from build123d import *

# Parameters (mm, degrees)
EXTRUDE_1_DEPTH      = 0.5
EXTRUDE_1_DEPTH_BACK = 0.5
SKETCH_1_R           = 0.6


with BuildPart() as part:
    # 草图1 → 凸台-拉伸1 (new, two sides: drawn at the far end of the back side and taken through both)
    with BuildSketch(Plane(origin=(0, 0, 0), x_dir=(0, 0, -1), z_dir=(1, 0, 0)).offset(-EXTRUDE_1_DEPTH_BACK)):
        with BuildLine():
            Line((-1.575903864, -5.685642181), (-0.792131706, -4.328108982))
            ThreePointArc((-0.792131706, -4.328108982), (-1.835210176, -2.355544978), (-3.685531471, -3.602674702))
            ThreePointArc((-3.685531471, -3.602674702), (0, 4.4), (3.685531471, -3.602674702))
            ThreePointArc((3.685531471, -3.602674702), (1.835210176, -2.355544978), (0.792131706, -4.328108982))
            Line((0.792131706, -4.328108982), (1.575903864, -5.685642181))
            ThreePointArc((1.575903864, -5.685642181), (0, 5.9), (-1.575903864, -5.685642181))
        make_face()
        with Locations((2.2, -3.810511777)):
            Circle(SKETCH_1_R, mode=Mode.SUBTRACT)
        with Locations((-2.2, -3.810511777)):
            Circle(SKETCH_1_R, mode=Mode.SUBTRACT)
    extrude(amount=EXTRUDE_1_DEPTH + EXTRUDE_1_DEPTH_BACK)


solid = part.part
Part model, mm, in its own coordinate system. A direction names the side the tool comes from. Give positions to 0.01 mm unless a question says otherwise; leave off trailing zeros. Order: outer loops, then holes, each group sorted by start corner. A loop starts at its lowest first (then second) coordinate and runs counter-clockwise, first axis right, second up. Notation, with made-up numbers: (-2, 34) - (36, 34) arc R24 cw to (36, 61) - close; hole circle Ø6 at (71.5, 34.5). An arc over 180 degrees is marked (long way). Use a Markdown table: item, result.
1) Two-plate mould, pull along Y, no slides. Class faces 3 (the cylindrical face through (-0.01, -4.34, 1.92)), 4 (the flat face through (-0.01, -5, -1.18)), 5 (the flat face through (0.5, -2.9, 1.3)): +Y half, -Y half, draft (parallel to the pull), parting line (faces both ways), or undercut.
Checked values:
| item | result |
|---|---|
| face 3 | undercut |
| face 4 | -Y half |
| face 5 | draft |
2) Saw through at A-A on y = 1. List the corners of the cut face in (x, z), plus the area to 3 significant figures.
Checked values:
| item | result |
|---|---|
| outline | (-0.5, -5.81) - (0.5, -5.81) - (0.5, -4.63) - (-0.5, -4.63) - close; (-0.5, 4.63) - (0.5, 4.63) - (0.5, 5.81) - (-0.5, 5.81) - close |
| area | 2.37 mm² |
3) Saw through at C-C on x = -0.15. List the corners of the cut face in (y, z), plus the area to 3 significant figures.
Checked values:
| item | result |
|---|---|
| outline | (-5.69, -1.58) arc R5.9 ccw (long way) to (-5.69, 1.58) - (-4.33, 0.79) arc R1.5 ccw (long way) to (-3.6, 3.69) arc R4.85 cw (long way) to (-3.6, -3.69) arc R1.5 ccw (long way) to (-4.33, -0.79) - close; hole circle Ø1.2 at (-3.81, -2.2); hole circle Ø1.2 at (-3.81, 2.2) |
| area | 43.0 mm² |
4) Saw through at B-B on z = 2.2. List the corners of the cut face in (x, y), plus the area to 3 significant figures.
Checked values:
| item | result |
|---|---|
| outline | (-0.5, -5.47) - (0.5, -5.47) - (0.5, -4.41) - (-0.5, -4.41) - close; (-0.5, -3.21) - (0.5, -3.21) - (0.5, -2.31) - (-0.5, -2.31) - close; (-0.5, 3.87) - (0.5, 3.87) - (0.5, 5.47) - (-0.5, 5.47) - close |
| area | 3.57 mm² |
5) Saw through at D-D on z = -3. List the corners of the cut face in (x, y), plus the area to 3 significant figures.
Checked values:
| item | result |
|---|---|
| outline | (-0.5, -5.08) - (0.5, -5.08) - (0.5, -2.54) - (-0.5, -2.54) - close; (-0.5, 3.36) - (0.5, 3.36) - (0.5, 5.08) - (-0.5, 5.08) - close |
| area | 4.26 mm² |
6) Probe L1, parallel to Y at x = -0.4, z = 2; L2, parallel to Z at x = 0.2, y = -4; L3, parallel to Z at x = -0.35, y = -2.5. List the from-to ranges inside material, lowest first. Write a range as from..to.
Checked values:
| item | result |
|---|---|
| L1 | -5.55..-4.38, -3.24..-2.32, 3.97..5.55 |
| L2 | -4.34..-2.77, -1.63..-0.71, 0.71..1.63, 2.77..4.34 |
| L3 | -5.34..-4.4, -2.93..-1.47, 1.47..2.93, 4.4..5.34 |
7) 3-axis set-ups, long thin cutter, end or side, ignore diameter. For faces 1 (the flat face through (-0.01, -5.02, 1.19)), 2 (the cylindrical face through (-0.01, -4.34, -2.48)): which of +Z, -Z, +X, -X, +Y, -Y reach the whole face in a straight line?
Checked values:
| item | result |
|---|---|
| face 1 | +X, -X, -Y |
| face 2 | +X, -X |
8) Flat gauge pins, fed straight in: P1, Ø3, axis at y = 2, z = 3, coming from the +X side; P2, Ø0.7, axis at y = -3.81, z = -2.2, coming from the +X side. Where does each tip first touch, or does it go through?
Checked values:
| item | result |
|---|---|
| P1 | x = 0.5 |
| P2 | through |
